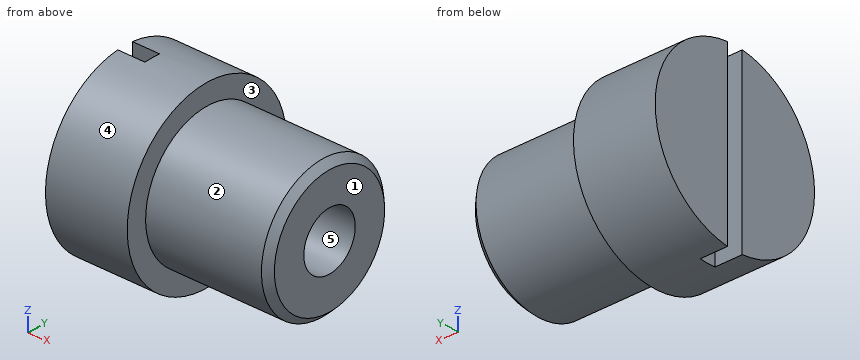
from build123d import *

# Parameters (mm, degrees)
SKETCH_2_R             = 5
EXTRUDE_1_DEPTH        = 9
SKETCH_5_R             = 6.5
EXTRUDE_2_DEPTH        = 6
SKETCH_6_W             = 30
SKETCH_6_H             = 1.2
CUT_EXTRUDE_1_DEPTH    = 2
HOLE_WIZARD_M5_1_D     = 4.2
HOLE_WIZARD_M5_1_DEPTH = 11
HOLE_WIZARD_M5_1_TIP   = 1.2618073
CHAMFER_1_SIZE         = 0.5


with BuildPart() as part:
    # 草图2 → 凸台-拉伸1 (new body)
    with BuildSketch(Plane(origin=(0, 0, 0), x_dir=(0, 0, -1), z_dir=(1, 0, 0))):
        Circle(SKETCH_2_R)
    extrude(amount=EXTRUDE_1_DEPTH)

    # 草图5 → 凸台-拉伸2 (add)
    with BuildSketch(Plane.ZY):
        Circle(SKETCH_5_R)
    extrude(amount=EXTRUDE_2_DEPTH)

    # 草图6 → 切除-拉伸1 (cut)
    with BuildSketch(Plane.ZY.offset(6)):
        Rectangle(SKETCH_6_W, SKETCH_6_H)
    extrude(amount=-CUT_EXTRUDE_1_DEPTH, mode=Mode.SUBTRACT)

    # M5 螺纹孔1
    with Locations(Plane(origin=(9, 0, 0), x_dir=(0, 0, 1), z_dir=(1, 0, 0))):
        with Locations((0, 0)):
            Hole(HOLE_WIZARD_M5_1_D / 2, depth=HOLE_WIZARD_M5_1_DEPTH)
            with Locations((0, 0, -(HOLE_WIZARD_M5_1_DEPTH + HOLE_WIZARD_M5_1_TIP / 2))):  # 118° drill point
                Cone(0, HOLE_WIZARD_M5_1_D / 2, HOLE_WIZARD_M5_1_TIP, mode=Mode.SUBTRACT)

    # 倒角1
    chamfer_1_edges = [part.edges().sort_by_distance(p)[0] for p in [
        (9, 0, 5),
    ]]
    chamfer(chamfer_1_edges, length=CHAMFER_1_SIZE)


solid = part.part
Can you work these out from the model? Positions are in its coordinate system, mm. Face numbers are marked on the shaded views. A direction names the side the tool comes from. Coordinates: 2 decimals unless noted, no trailing zeros. Loops run counter-clockwise (first coordinate to the right, second up) from the corner with the lowest first, then second, coordinate; pieces in that order, holes last. Notation, with made-up numbers: (-27, 41) - (8, 41) arc R15 cw to (8, 46) - close; hole circle Ø8 at (87, 88.5). An arc over 180 degrees is marked (long way). Answer as a JSON object with one key per item and string values. Group by question number.
Item 1: If we section it at B-B (x = -1.25): List the corners of the cut face in (y, z) for me.
Item 2: For pin 1 (1 mm diameter, centred on x = 2, y = 0, fed in from +Z); pin 2 (0.6 mm diameter, centred on x = -5, z = -0.5, fed in from -Y); pin 3 (1 mm diameter, centred on x = -4.5, z = -1, fed in from +Y), each with a flat end and sliding along its axis, tell me the tip position at first contact or that it passes through.
Item 3: On a 3-axis mill with a long thin cutter (end or side, diameter ignored), from which of +Z, -Z, +X, -X, +Y, -Y can I reach the whole of each face in a straight line? I mean the marked faces 1 and 2. Say none if no direction works.
Item 4: If we section it at C-C (y = -5.25): List the corners of the cut face in (x, z) for me, plus the area to 3 significant figures.
Item 5: If we mould it in two halves opening along Z, with no side actions, what happens to the marked faces 3, 4 and 5? For each: released by +Z, released by -Z, zero draft, split by the parting line, or undercut.
Item 6: If we section it at A-A (x = 8.25): List the corners of the cut face in (y, z) for me, plus the area to 3 significant figures.
Item 7: If I drill on L1, parallel to Y at x = 2.75, z = 0; L2, parallel to Y at x = 3.75, z = 1.5; L3, parallel to X at y = -1.5, z = 5.5, over which ranges is the centre line in solid material (lowest first)? Write a range as from..to.
Returned:
{
 "1": {"outline": "circle Ø13 at (0, 0); hole circle Ø4.2 at (0, 0)"},
 "2": {"pin 1": "stops at z = 5", "pin 2": "stops at y = -6.5", "pin 3": "stops at y = 6.48"},
 "3": {"face 1": "+Z, -Z, +X, +Y, -Y", "face 2": "+X"},
 "4": {"outline": "(-6, -3.83) - (0, -3.83) - (0, 3.83) - (-6, 3.83) - close", "area": "46.0 mm²"},
 "5": {"face 3": "zero draft", "face 4": "split by the parting line", "face 5": "undercut"},
 "6": {"outline": "circle Ø10 at (0, 0); hole circle Ø4.2 at (0, 0)", "area": "64.7 mm²"},
 "7": {"L1": "y = -5..-2.1, 2.1..5", "L2": "y = -4.77..-1.47, 1.47..4.77", "L3": "x = -6..0"}
}
